from build123d import *

# Parameters (mm, degrees)
SKETCH_1_W             = 80
SKETCH_1_H             = 39
EXTRUDE_1_DEPTH        = 14
HOLE_WIZARD_M6_1_D     = 5
HOLE_WIZARD_M6_1_DEPTH = 17
HOLE_WIZARD_M6_1_TIP   = 1.502151548
HOLE_WIZARD_M6_2_D     = 5
HOLE_WIZARD_M6_2_DEPTH = 17
HOLE_WIZARD_M6_2_TIP   = 1.502151548


with BuildPart() as part:
    # 草图1 → 凸台-拉伸1 (new body)
    with BuildSketch(Plane.XY):
        Rectangle(SKETCH_1_W, SKETCH_1_H)
    extrude(amount=EXTRUDE_1_DEPTH)

    # M6 螺纹孔1
    with Locations(Plane(origin=(0, -19.5, 0), x_dir=(-1, 0, 0), z_dir=(0, -1, 0))):
        with Locations((-21, -7), (21, -7)):
            Hole(HOLE_WIZARD_M6_1_D / 2, depth=HOLE_WIZARD_M6_1_DEPTH)
            with Locations((0, 0, -(HOLE_WIZARD_M6_1_DEPTH + HOLE_WIZARD_M6_1_TIP / 2))):  # 118° drill point
                Cone(0, HOLE_WIZARD_M6_1_D / 2, HOLE_WIZARD_M6_1_TIP, mode=Mode.SUBTRACT)

    # M6 螺纹孔2
    with Locations(Plane(origin=(0, 19.5, 0), x_dir=(1, 0, 0), z_dir=(0, 1, 0))):
        with Locations((-33, -7), (33, -7)):
            Hole(HOLE_WIZARD_M6_2_D / 2, depth=HOLE_WIZARD_M6_2_DEPTH)
            with Locations((0, 0, -(HOLE_WIZARD_M6_2_DEPTH + HOLE_WIZARD_M6_2_TIP / 2))):  # 118° drill point
                Cone(0, HOLE_WIZARD_M6_2_D / 2, HOLE_WIZARD_M6_2_TIP, mode=Mode.SUBTRACT)


solid = part.part
The model under review builds one solid part; all positions refer to its coordinate system, in mm. A direction names the side the tool comes from. Round coordinates to 2 decimals unless told otherwise and drop trailing zeros. Order: outer loops, then holes, each group sorted by start corner. A loop starts at its lowest first (then second) coordinate and runs counter-clockwise, first axis right, second up. Notation, with made-up numbers: (-23.5, 32.25) -> (-11.5, 32.25) arc R3 ccw to (-11.5, 37.25) -> close; hole circle Ø11 at (9, 23). An arc over 180 degrees is marked (long way). Use CSV: the item, a comma, the result in double quotes. Start each with the question number.
(1) Tool access review of faces 1 (the face through (35.5, 10.9, 6.9)), 2 (the face through (-40, 0, 7)), 3 (the face through (18.5, -10.9, 6.9)): name each direction out of +Z, -Z, +X, -X, +Y, -Y from which nothing blocks a thin tool from reaching the whole face with its end or side.
(2) Wall thickness on probe 1 along Z at (x, y) = (-33, 11.75); probe 2 along X at (y, z) = (-9, 7.5); probe 3 along X at (y, z) = (17, 8): over which ranges is each line inside the solid? List them lowest first. Write a range as from..to.
(3) Mouldability with a two-part tool opening along X and no side actions: class faces 4 (the face through (-1, 0, 0)), 5 (the face through (-35.31, 10.88, 7.96)), 6 (the face through (40, 0, 7)) as pulls with the +X half, pulls with the -X half, needs draft (parallel to the pull), parting line crosses it, or undercut.
(4) Consider section A-A on y = -14. Write out the cut boundary in (x, z).
Responses:
1,face 1,"+Y"
1,face 2,"+Z, -Z, -X, +Y, -Y"
1,face 3,"-Y"
2,probe 1,"0..4.5, 9.5..14"
2,probe 2,"-40..-23.45, -18.55..18.55, 23.45..40"
2,probe 3,"-40..-35.29, -30.71..30.71, 35.29..40"
3,face 4,"needs draft"
3,face 5,"undercut"
3,face 6,"pulls with the +X half"
4,outline,"(-40, 0) -> (40, 0) -> (40, 14) -> (-40, 14) -> close; hole circle Ø5 at (-21, 7); hole circle Ø5 at (21, 7)"
